Work out the finished part from the listing and answer in its coordinate system (mm). Coordinates: 2 decimals unless noted, no trailing zeros. Order: outer loops, then holes, each group sorted by start corner. A loop starts at its lowest first (then second) coordinate and runs counter-clockwise, first axis right, second up.
1. The part is cut by section B-B, the plane y = -2.25. Give the vertices of the cut face in (x, z).
2. Flat-ended cylindrical pins translate along their axes: pin 1 Ø6 at (x, y) = (49.5, 5) entering from -Z; pin 2 Ø4 at (y, z) = (-2, -11.5) entering from -X; pin 3 Ø5 at (x, y) = (15, 1.5) entering from +Z; pin 4 Ø7 at (x, z) = (-157.5, 0) entering from +Y. Find the tip coordinate at first contact, or state that the pin passes through.
3. The part is cut by section C-C, the plane x = 157.5. Give the vertices of the cut face in (y, z), then the cut area to 3 significant figures.
4. The part is cut by section A-A, the plane z = 0. Give the vertices of the cut face in (x, y).
5. Find the intervals of material crossed by probe 1 along X at (y, z) = (-1.5, 0); probe 2 along Z at (x, y) = (10, 2); probe 3 along Y at (x, z) = (-110.5, 19.5), in increasing order.
6. The part is cut by section D-D, the plane x = -27.5. Give the vertices of the cut face in (y, z), then the cut area to 3 significant figures.
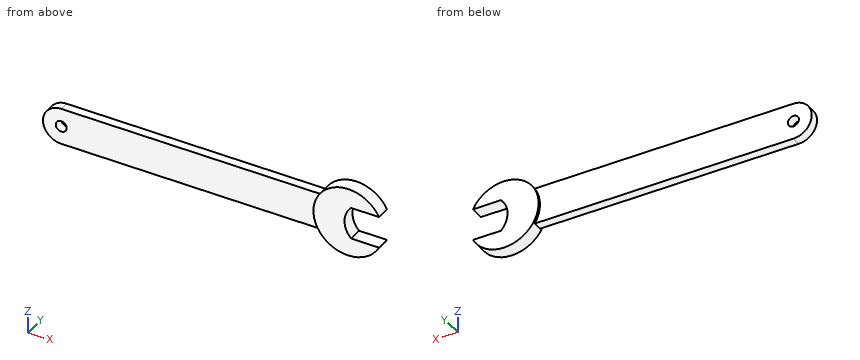
```python
from build123d import *

# Parameters (mm, degrees)
WRENCH_OUTLINE_SKETCH_R  = 6
WRENCH_HANDLE_10MM_DEPTH = 5
JAW_HEAD_BOSS_15MM_DEPTH = 7.5


with BuildPart() as part:
    # Wrench Outline Sketch → Wrench Handle 10mm (new, symmetric)
    with BuildSketch(Plane(origin=(0, 0, 0), x_dir=(1, 0, 0), z_dir=(0, 1, 0))):
        with BuildLine():
            Line((125.189011157, 20), (-157.5, 20))
            ThreePointArc((-157.5, 20), (-177.5, 0), (-157.5, -20))
            Line((-157.5, -20), (125.189011157, -20))
            ThreePointArc((125.189011157, -20), (119.5, 0), (125.189011157, 20))
        make_face()
        with Locations(Location((-157.5, 0, 0), (0, 0, 270))):
            Circle(WRENCH_OUTLINE_SKETCH_R, mode=Mode.SUBTRACT)
    extrude(amount=WRENCH_HANDLE_10MM_DEPTH, both=True)

    # Jaw Head Sketch → Jaw Head Boss 15mm (add, symmetric)
    with BuildSketch(Plane(origin=(0, 0, 0), x_dir=(1, 0, 0), z_dir=(0, 1, 0))):
        with BuildLine():
            Line((160.646428929, -17.5), (191.230549951, -17.5))
            ThreePointArc((191.230549951, -17.5), (119.5, 0), (191.230549951, 17.5))
            Line((191.230549951, 17.5), (160.646428929, 17.5))
            ThreePointArc((160.646428929, 17.5), (153.5, 0), (160.646428929, -17.5))
        make_face()
    extrude(amount=JAW_HEAD_BOSS_15MM_DEPTH, both=True)


solid = part.part
```
Geometry says:
1. outline: (-157.5, -20) - (125.19, -20) arc R38 ccw to (191.23, -17.5) - (160.65, -17.5) arc R25 cw to (160.65, 17.5) - (191.23, 17.5) arc R38 ccw to (125.19, 20) - (-157.5, 20) arc R20 ccw to start; hole circle Ø12 at (-157.5, 0)
2. pin 1: stops at z = -20
2. pin 2: stops at x = -175.1
2. pin 3: stops at z = 20
2. pin 4: passes through
3. outline: (-7.5, -38) - (7.5, -38) - (7.5, -13.56) - (-7.5, -13.56) - close; (-7.5, 13.56) - (7.5, 13.56) - (7.5, 38) - (-7.5, 38) - close
3. area: 733 mm2
4. outline: (-177.5, -5) - (-163.5, -5) - (-163.5, 5) - (-177.5, 5) - close; (-151.5, -5) - (119.5, -5) - (119.5, -7.5) - (153.5, -7.5) - (153.5, 7.5) - (119.5, 7.5) - (119.5, 5) - (-151.5, 5) - close
5. probe 1: x = -177.5 to -163.5, -151.5 to 153.5
5. probe 2: z = -20 to 20
5. probe 3: y = -5 to 5
6. outline: (-5, -20) - (5, -20) - (5, 20) - (-5, 20) - close
6. area: 400 mm2
